Can you work these out from the model? Positions are in its coordinate system, mm. Face numbers are marked on the shaded views. A direction names the side the tool comes from. Coordinates: 2 decimals unless noted, no trailing zeros. Loops run counter-clockwise (first coordinate to the right, second up) from the corner with the lowest first, then second, coordinate; pieces in that order, holes last. Notation, with made-up numbers: (31, -25.5) - (47, -25.5) arc R16 cw to (47, -16.5) - close; hole circle Ø9 at (43, 53.25). An arc over 180 degrees is marked (long way). Put each result on its own line as item: value. Start each with the question number.
from build123d import *

# Parameters (mm, degrees)
CUT_EXTRUDE_1_DEPTH      = 2
CUT_EXTRUDE_1_DEPTH_BACK = 2


with BuildPart() as part:
    # 草图1 → 旋转1 (revolve)
    with BuildSketch(Plane.XY, mode=Mode.PRIVATE) as revolve_1_sk:
        with BuildLine():
            Line((0, 25.8), (3.5, 25.8))
            ThreePointArc((3.5, 25.8), (3.853553391, 25.653553391), (4, 25.3))
            Line((4, 25.3), (4, 12.9))
            Line((4, 12.9), (5, 12.9))
            Line((5, 12.9), (5, 0.5))
            Line((5, 0.5), (4.5, 0))
            Line((4.5, 0), (2.5, 0))
            Line((2.5, 0), (2.5, -31.5095))
            Line((2.5, -31.5095), (2.0095, -32))
            Line((2.0095, -32), (0, -32))
            Line((0, -32), (0, 25.8))
        make_face()
    revolve(revolve_1_sk.sketch.rotate(Axis((0, -32, 0), (0, 1, 0)), 270), axis=Axis((0, -32, 0), (0, 1, 0)))

    # 草图2 → 切除-拉伸1 (cut, two sides: drawn at the far end of the back side and taken through both)
    with BuildSketch(Plane(origin=(0, 25.8, 0), x_dir=(-1, 0, 0), z_dir=(0, 1, 0)).offset(-CUT_EXTRUDE_1_DEPTH_BACK)):
        Polygon((1.5, -0.866025404), (1.5, 0.866025404), (0, 1.732050808), (-1.5, 0.866025404), (-1.5, -0.866025404), (0, -1.732050808), align=None)
    extrude(amount=CUT_EXTRUDE_1_DEPTH + CUT_EXTRUDE_1_DEPTH_BACK, mode=Mode.SUBTRACT)

    # 草图3 → 切除-旋转1 (revolve, cut)
    with BuildSketch(Plane.XY, mode=Mode.PRIVATE) as cut_revolve_1_sk:
        Polygon((0, 25.8), (1.5, 25.8), (1.5, 23.8), (0, 22.933974596), align=None)
    revolve(cut_revolve_1_sk.sketch.rotate(Axis((0, 22.933974596, 0), (0, 1, 0)), 270), axis=Axis((0, 22.933974596, 0), (0, 1, 0)), mode=Mode.SUBTRACT)


solid = part.part
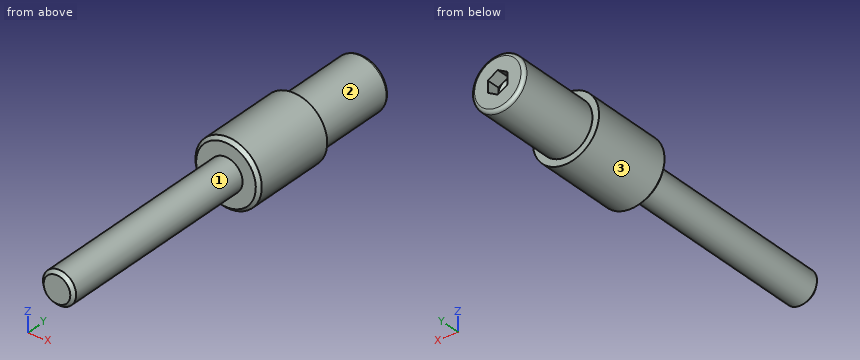
Q1. I want a section at A-A on y = 14.5. List the corners of the cut face in (x, z) for me, and give its area (3 significant figures).
Q2. Will these pins go through, and if not, where does the flat tip stop? pin 1 (4 mm diameter, centred on y = 15, z = 1.5, fed in from -X); pin 2 (3 mm diameter, centred on y = -21, z = -2, fed in from +X); pin 3 (4 mm diameter, centred on y = 8.5, z = -3.5, fed in from -X); pin 4 (2 mm diameter, centred on x = 4, y = -20, fed in from +Z).
Q3. Please list where these lines run through material, in increasing order: line 1 along Y through (x, z) = (-0.5, 2.75); line 2 along X through (y, z) = (-1.5, -2); line 3 along X through (y, z) = (-12, -1.5). Write a range as [from, to].
Q4. I want a section at B-B on y = -25. List the corners of the cut face in (x, z) for me.
Q5. On a 3-axis mill with a long thin cutter (end or side, diameter ignored), from which of +Z, -Z, +X, -X, +Y, -Y can I reach the whole of each face in a straight line? I mean the marked faces 1, 2 and 3. Say none if no direction works.
Calculated:
1. outline: circle Ø8 at (0, 0)
1. area: 50.3 mm2
2. pin 1: x = -4
2. pin 2: x = 2.45
2. pin 3: x = -4.77
2. pin 4: through
3. line 1: [0, 25.8]
3. line 2: [-1.5, 1.5]
3. line 3: [-2, 2]
4. outline: circle Ø5 at (0, 0)
5. face 1: -Y
5. face 2: +Y
5. face 3: +Y, -Y
